Build history of the part. All positions in model axes, mm. Face numbers are marked on the shaded views. A direction names the side the tool comes from. Give positions to 0.01 mm unless a question says otherwise; leave off trailing zeros. Loops run counter-clockwise (first coordinate to the right, second up) from the corner with the lowest first, then second, coordinate; pieces in that order, holes last. Notation, with made-up numbers: M 31,32.5 L 77,32.5 A9 cw 77,42.5 Z; hole C 20.5,20.25 d2. An arc over 180 degrees is marked long. Answer in a Markdown table with one row per item. Add a question column.
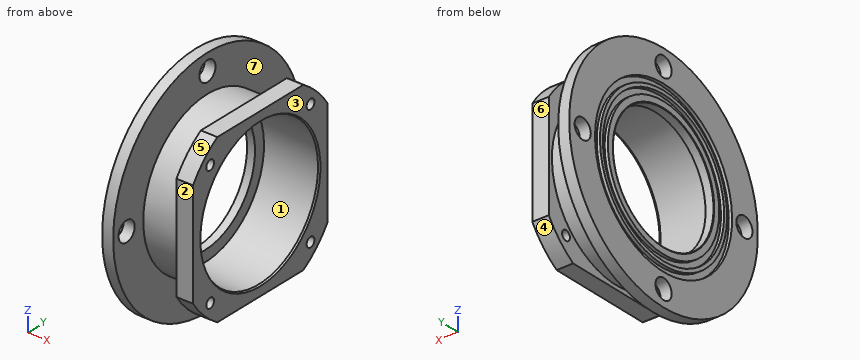
```python
from build123d import *

# Parameters (mm, degrees)
SKETCH5_R          = 152.5
SKETCH5_R_2        = 141.5
CUT_EXTRUDE1_DEPTH = 5.9
SKETCH6_R          = 135
SKETCH6_R_2        = 124
CUT_EXTRUDE2_DEPTH = 5.9
SKETCH7_R          = 18
CUT_EXTRUDE3_DEPTH = 20
CIRPATTERN1_COUNT  = 4
CIRPATTERN2_COUNT  = 4
CUT_EXTRUDE4_DEPTH = 30
CHAMFER1_SIZE      = 3
CHAMFER1_SIZE2     = 1.732050808
CHAMFER2_SIZE      = 1
CHAMFER2_SIZE2     = 0.577350269


with BuildPart() as part:
    # Sketch4 → Revolve1 (revolve)
    with BuildSketch(Plane.XY, mode=Mode.PRIVATE) as revolve1_sk:
        Polygon((-62.794117647, 112), (-62.794117647, 210), (-42.794117647, 210), (-42.794117647, 143), (23.205882353, 143), (23.205882353, 178), (53.205882353, 178), (53.205882353, 132), (-47.794117647, 132), (-47.794117647, 112), align=None)
    revolve(revolve1_sk.sketch.rotate(Axis((-131.764705882, 0, 0), (1, 0, 0)), 90), axis=Axis((-131.764705882, 0, 0), (1, 0, 0)))

    # Sketch5 → Cut-Extrude1 (cut)
    with BuildSketch(Plane.ZY.offset(62.794117647)):
        Circle(SKETCH5_R)
        Circle(SKETCH5_R_2, mode=Mode.SUBTRACT)
    extrude(amount=-CUT_EXTRUDE1_DEPTH, mode=Mode.SUBTRACT)

    # Sketch6 → Cut-Extrude2 (cut)
    with BuildSketch(Plane.ZY.offset(62.794117647)):
        Circle(SKETCH6_R)
        Circle(SKETCH6_R_2, mode=Mode.SUBTRACT)
    extrude(amount=-CUT_EXTRUDE2_DEPTH, mode=Mode.SUBTRACT)

    # Sketch7 → Cut-Extrude3 (cut)
    with BuildSketch(Plane.ZY.offset(62.794117647)):
        with Locations((0, 180)):
            Circle(SKETCH7_R)
    cut_extrude3 = extrude(amount=-CUT_EXTRUDE3_DEPTH, mode=Mode.SUBTRACT)

    # CirPattern1: Cut-Extrude3 ×4 about axis
    cirpattern1_axis = Axis((0, 0, 0), (1, 0, 0))
    for i in range(1, CIRPATTERN1_COUNT):
        add(cut_extrude3.rotate(cirpattern1_axis, i * 360 / CIRPATTERN1_COUNT), mode=Mode.SUBTRACT)

    # Sketch9 → M20 Tapped Hole1 (revolve, cut)
    with BuildSketch(Plane(origin=(53.205882353, 111.722871427, -111.722871427), x_dir=(0, 0, -1), z_dir=(0, 1, 0))):
        Polygon((0, 0), (0, 57.757530416), (8.75, 52.5), (8.75, 0), align=None)
    m20_tapped_hole1 = revolve(axis=Axis((59.555882353, 111.722871427, -111.722871427), (-1, 0, 0)), mode=Mode.SUBTRACT)

    # CirPattern2: M20 Tapped Hole1 ×4 about axis
    cirpattern2_axis = Axis((0, 0, 0), (1, 0, 0))
    for i in range(1, CIRPATTERN2_COUNT):
        add(m20_tapped_hole1.rotate(cirpattern2_axis, i * 360 / CIRPATTERN2_COUNT), mode=Mode.SUBTRACT)

    # Sketch12 → Cut-Extrude4 (cut)
    with BuildSketch(Plane(origin=(53.205882353, 0, 0), x_dir=(0, 0, -1), z_dir=(1, 0, 0))):
        with BuildLine():
            Line((-95.833188406, 150), (95.833188406, 150))
            ThreePointArc((95.833188406, 150), (0, 178), (-95.833188406, 150))
        make_face()
        with BuildLine():
            Line((-150, 95.833188406), (-150, -95.833188406))
            ThreePointArc((-150, -95.833188406), (-178, 0), (-150, 95.833188406))
        make_face()
        with BuildLine():
            Line((-95.833188406, -150), (95.833188406, -150))
            ThreePointArc((95.833188406, -150), (0, -178), (-95.833188406, -150))
        make_face()
        with BuildLine():
            Line((150, 95.833188406), (150, -95.833188406))
            ThreePointArc((150, -95.833188406), (178, 0), (150, 95.833188406))
        make_face()
    extrude(amount=-CUT_EXTRUDE4_DEPTH, mode=Mode.SUBTRACT)

    # Chamfer1
    chamfer1_edges = [part.edges().sort_by_distance(p)[0] for p in [
        (53.205882353, 0, -132),
    ]]
    chamfer1_side = [part.faces().sort_by_distance(p)[0] for p in [
        (2.705882353, 0, -132),
    ]]
    chamfer(chamfer1_edges, length=CHAMFER1_SIZE, length2=CHAMFER1_SIZE2, reference=chamfer1_side[0])

    # Chamfer2
    chamfer2_edges = [part.edges().sort_by_distance(p)[0] for p in [
        (-62.794117647, 0, -112),
    ]]
    chamfer2_side = [part.faces().sort_by_distance(p)[0] for p in [
        (-62.794117647, 0, -120.492750365),
    ]]
    chamfer(chamfer2_edges, length=CHAMFER2_SIZE, length2=CHAMFER2_SIZE2, reference=chamfer2_side[0])


solid = part.part
```
(1) Pin check, flat tips, straight feed: pin 1 (24 mm diameter, centred on x = 45.5, y = 30.5, fed in from +Z); pin 2 (5 mm diameter, centred on x = 24.5, z = 64, fed in from -Y); pin 3 (5 mm diameter, centred on x = -50, y = -129.5, fed in from -Z); pin 4 (12 mm diameter, centred on y = -110.5, z = -115.5, fed in from +X). Stop position of each tip, or through.
(2) Wall check: line 1 (Y direction, x = -52.25, z = 0); line 2 (X direction, y = 135.5, z = -96); line 3 (Y direction, x = 8, z = -5.5). Give the ranges that are in metal, low to high.
(3) Slice it at D-D, the plane x = 13.5. Give the cut face in (y, z), then the cut area to 3 significant figures.
(4) Pull direction Y, two halves, no side cores. Call the marked faces 1, 2, 3 and 4: +Y half, -Y half, draft (parallel to the pull), parting line (faces both ways), or undercut.
(5) Tool access for the marked faces 5, 6 and 7: list every direction of +Z, -Z, +X, -X, +Y, -Y with a clear straight run to the whole face (end or side of a thin tool).
(6) Slice it at A-A, the plane z = -180. Give the cut face in (x, y).
(7) Slice it at C-C, the plane z = 0. State how many separate pieces and enclosed holes the cut face has, then the cut area to 3 significant figures.
Solution:
| question | item | result |
|---|---|---|
| 1 | pin 1 | z = 150 |
| 1 | pin 2 | y = -150 |
| 1 | pin 3 | z = -167.25 |
| 1 | pin 4 | x = 53.21 |
| 2 | line 1 | -210 to -198, -162 to -112, 112 to 162, 198 to 210 |
| 2 | line 2 | -62.79 to -42.79, 23.21 to 53.21 |
| 2 | line 3 | -142.89 to -131.89, 131.89 to 142.89 |
| 3 | outline | C 0,0 d286; hole C 0,0 d264 |
| 3 | area | 9,500 mm^2 |
| 4 | face 1 | undercut |
| 4 | face 2 | -Y half |
| 4 | face 3 | draft |
| 4 | face 4 | +Y half |
| 5 | face 5 | +Z, +X, -Y |
| 5 | face 6 | +Z, -Z, +X, +Y |
| 5 | face 7 | none |
| 6 | outline | M -62.79,-108.17 L -42.79,-108.17 L -42.79,-18 L -62.79,-18 Z; M -62.79,18 L -42.79,18 L -42.79,108.17 L -62.79,108.17 Z |
| 7 | separate pieces | 4 |
| 7 | enclosed holes | 0 |
| 7 | area | 4,550 mm^2 |
